```python
from build123d import *

# Parameters (mm, degrees)
SWEEP_THIN1_PROFILE_R   = 15
SWEEP_THIN1_PROFILE_R_2 = 13


with BuildPart() as part:
    # Sweep-Thin1: sweep along a curve in space
    with BuildLine() as sweep_thin1_path:
        Line((19403.083026604, -840, -3659.86490803), (19403.083026604, -807.464377163, -3659.86490803))
        ThreePointArc((19403.083026604, -807.464377163, -3659.86490803), (19403.083026604, -790.016622217, -3659.484196663), (19403.083026604, -772.602080064, -3658.342787267))
        Line((19403.083026604, -772.602080064, -3658.342787267), (19403.083026604, 756.627756068, -3524.552512679))
        ThreePointArc((19403.083026604, 756.627756068, -3524.552512679), (19403.083026604, 774.042298221, -3523.411103283), (19403.083026604, 791.490053167, -3523.030391916))
        Line((19403.083026604, 791.490053167, -3523.030391916), (19403.083026604, 854.025676004, -3523.030391916))
    # Sweep-Thin1 profile (on start of the path) → Sweep-Thin1 (sweep)
    with BuildSketch(Plane(origin=(19403.083026604, -840, -3659.86490803), x_dir=(0, 0, 1), z_dir=(0, 1, 0))):
        Circle(SWEEP_THIN1_PROFILE_R)
        Circle(SWEEP_THIN1_PROFILE_R_2, mode=Mode.SUBTRACT)
    sweep(path=sweep_thin1_path.line)


solid = part.part
```
Work out the finished part from the listing and answer in its coordinate system (mm). A direction names the side the tool comes from. Round coordinates to 2 decimals unless told otherwise and drop trailing zeros. Write each loop counter-clockwise with the first axis right and the second up, starting at its lowest first coordinate (ties: lowest second). Pieces come first, ordered by that corner, then holes. Notation, with made-up numbers: (16.25, -31) -> (32.25, -31) arc R33 cw to (32.25, 7) -> close; hole circle Ø3 at (-7.5, -39). An arc over 180 degrees is marked (long way). Write each question's results on one line, items separated by ' | '.
Q1. Which of the six approach directions +Z, -Z, +X, -X, +Y, -Y give full straight-line access (tool end or side, diameter ignored) to faces 1 (the cylindrical face through (19388.44, 823.2, -3526.28)), 2 (the cylindrical face through (19398.1, -823.5, -3647.86)), 3 (the flat face through (19416.5, 854.026, -3523.1))?
Data:
face 1: +Y | face 2: -Y | face 3: +Z, -Z, +X, -X, +Y
Q2. Straight lines are drawn through the part: line 1 along X through (y, z) = (613, -3540); line 2 along Z through (x, y) = (19399, 9); line 3 along X through (y, z) = (82.5, -3575.5). For each, find the intervals that lie inside material, in ascending order. Write a range as [from, to].
Data:
line 1: [19388.36, 19390.4], [19415.76, 19417.81] | line 2: [-3604.45, -3602.35], [-3577.57, -3575.47] | line 3: [19390.39, 19392.84], [19413.33, 19415.77]
Q3. Flat-ended cylindrical pins translate along their axes: P1, Ø1, axis at x = 19398, y = 662.5, coming from the +Z side; P2, Ø2, axis at x = 19409, y = 612.5, coming from the -Z side. Find the tip coordinate at first contact, or state that the pin passes through.
Data:
P1: z = -3518.44 | P2: z = -3551.4
Q4. Determine the mould class of faces 4 (the cylindrical face through (19398.1, 1.67, -3578.55)), 5 (the cylindrical face through (19388.44, 3, -3593.75)), 6 (the flat face through (19416.5, -840, -3659.9)), 7 (the cylindrical face through (19398.104, 823.196, -3511.022)) for opening direction Z: released by +Z, released by -Z, zero draft, split by the parting line, or undercut.
Data:
face 4: undercut | face 5: split by the parting line | face 6: zero draft | face 7: undercut
Q5. Section A-A, the plane x = 19395.5 is taken. Write down the section's boundary in (y, z).
Data:
outline: (-840, -3672.81) -> (-807.46, -3672.81) arc R412.94 ccw to (-771.47, -3671.24) -> (757.76, -3537.45) arc R387.06 cw to (791.49, -3535.97) -> (854.03, -3535.97) -> (854.03, -3533.59) -> (791.49, -3533.59) arc R389.44 ccw to (757.55, -3535.07) -> (-771.68, -3668.86) arc R410.56 cw to (-807.46, -3670.42) -> (-840, -3670.42) -> close; (-840, -3649.31) -> (-807.46, -3649.31) arc R389.44 ccw to (-773.52, -3647.82) -> (755.71, -3514.03) arc R410.56 cw to (791.49, -3512.47) -> (854.03, -3512.47) -> (854.03, -3510.09) -> (791.49, -3510.09) arc R412.94 ccw to (755.5, -3511.66) -> (-773.73, -3645.45) arc R387.06 cw to (-807.46, -3646.92) -> (-840, -3646.92) -> close
